Source: CAD feature listing. Evaluate the final solid. Frame: model axes, mm. A direction names the side the tool comes from. Round coordinates to 2 decimals unless told otherwise and drop trailing zeros. Order: outer loops, then holes, each group sorted by start corner. A loop starts at its lowest first (then second) coordinate and runs counter-clockwise, first axis right, second up. Notation, with made-up numbers: (87, 38.5) -> (125, 38.5) arc R19 ccw to (125, 59.5) -> close; hole circle Ø4 at (-3, 65). An arc over 180 degrees is marked (long way). Use a Markdown table: item, result. Add a question column.
```python
from build123d import *

# Parameters (mm, degrees)
CUT_EXTRUDE3_START = 95.1
CUT_EXTRUDE3_DEPTH = 26.1
CIRPATTERN1_COUNT  = 3


with BuildPart() as part:
    # Sketch2 → Revolve1 (revolve)
    with BuildSketch(Plane(origin=(0, 0, 0), x_dir=(0, 0, -1), z_dir=(1, 0, 0)), mode=Mode.PRIVATE) as revolve1_sk:
        Polygon((-172, 135), (172, 135), (172, 120), (426, 120), (426, 0), (0, 0), (-426, 0), (-426, 120), (-172, 120), align=None)
    revolve(revolve1_sk.sketch.rotate(Axis((0, 0, 564.378028921), (0, 0, -1)), 180), axis=Axis((0, 0, 564.378028921), (0, 0, -1)))

    # Sketch3 → Revolve2 (revolve)
    with BuildSketch(Plane(origin=(0, 0, 0), x_dir=(0, 0, -1), z_dir=(1, 0, 0)), mode=Mode.PRIVATE) as revolve2_sk:
        Polygon((426, -119), (426, -15), (923, -15), (923, -95), (678, -95), (678, -110), (614, -110), (614, -107), (602, -107), (602, -112.85), (454, -119), align=None)
    revolve2 = revolve(revolve2_sk.sketch.rotate(Axis((0, -15, 0), (0, 0, -1)), 270), axis=Axis((0, -15, 0), (0, 0, -1)))

    # Mirror1: Revolve2 across plane
    add(revolve2.mirror(Plane.XY))

    # Sketch5 → Cut-Extrude3 (cut)
    with BuildSketch(Plane(origin=(0, 0, 0), x_dir=(1, 0, 0), z_dir=(0, 1, 0)).offset(CUT_EXTRUDE3_START)):
        with BuildLine():
            Line((9, 742), (9, 614))
            ThreePointArc((9, 614), (0, 605), (-9, 614))
            Line((-9, 614), (-9, 742))
            ThreePointArc((-9, 742), (0, 751), (9, 742))
        make_face()
    cut_extrude3 = extrude(amount=-CUT_EXTRUDE3_DEPTH, mode=Mode.SUBTRACT)

    # Mirror2: Cut-Extrude3 across plane
    add(cut_extrude3.mirror(Plane.XY), mode=Mode.SUBTRACT)

    # Sketch7 → M16 Tapped Hole1 (revolve, cut)
    with BuildSketch(Plane(origin=(-51.961524227, 15, -923), x_dir=(0, 1, 0), z_dir=(1, 0, 0))):
        Polygon((0, 0), (0, 42.206024333), (7, 38), (7, 0), align=None)
    m16_tapped_hole1 = revolve(axis=Axis((-51.961524227, 15, -929.35), (0, 0, 1)), mode=Mode.SUBTRACT)

    # CirPattern1: M16 Tapped Hole1 ×3 about axis
    cirpattern1_axis = Axis((0, -15, 0), (0, 0, 1))
    for i in range(1, CIRPATTERN1_COUNT):
        add(m16_tapped_hole1.rotate(cirpattern1_axis, i * 360 / CIRPATTERN1_COUNT), mode=Mode.SUBTRACT)

    # Mirror3: M16 Tapped Hole1 across plane
    add(m16_tapped_hole1.mirror(Plane.XY), mode=Mode.SUBTRACT)

    # Mirror3 copy 1 sketch → Mirror3 copy 1 (revolve, cut)
    with BuildSketch(Plane(origin=(0, -75, 923), x_dir=(-0.8660254037844387, -0.4999999999999998, 0), z_dir=(-0.4999999999999998, 0.8660254037844387, 0))):
        Polygon((0, 0), (0, -42.206024333), (7, -38), (7, 0), align=None)
    revolve(axis=Axis((0, -75, 929.35), (0, 0, 1)), mode=Mode.SUBTRACT)

    # Mirror3 copy 2 sketch → Mirror3 copy 2 (revolve, cut)
    with BuildSketch(Plane(origin=(51.961524227, 15, 923), x_dir=(0.8660254037844384, -0.5000000000000004, 0), z_dir=(-0.5000000000000004, -0.8660254037844384, 0))):
        Polygon((0, 0), (0, -42.206024333), (7, -38), (7, 0), align=None)
    revolve(axis=Axis((51.961524227, 15, 929.35), (0, 0, 1)), mode=Mode.SUBTRACT)


solid = part.part
```
1) Reachability of faces 1 (the cylindrical face through (43.008, -82.456, 798.785)), 2 (the flat face through (-72, 43, -602)), 3 (the flat face through (1, -16, -923)), 4 (the cylindrical face through (-101.184, -64.511, -300.778)) from +Z, -Z, +X, -X, +Y, -Y: full face, straight path, thin tool, end or side. Return the list, or none.
2) Line query: probe 1 along X at (y, z) = (15, -901); probe 2 along Y at (x, z) = (0, -898.5); probe 3 along Y at (x, z) = (7, -52). Output: solid intervals per line, ascending. Write a range as from..to.
3) Section A-A on z = -732.5. Output: boundary loops of the cut face in (x, y), then the cut area to 3 significant figures.
4) Draft query along Z for faces 5 (the flat face through (-0.6, 89.4, -426)), 6 (the cylindrical face through (-82.531, 48.282, 439.804)), 7 (the flat face through (-36, -100, -614)). Return one class per face: pulls with the +Z half, pulls with the -Z half, needs draft (parallel to the pull), parting line crosses it, or undercut.
5) First-contact query: pin 1 Ø14.5 at (x, z) = (0.5, -637) entering from +Y; pin 2 Ø5.5 at (y, z) = (74, 637.5) entering from -X; pin 3 Ø11 at (x, y) = (0, -75) entering from -Z. Flat tips, straight axial feed; report the tip coordinate or a pass-through.
6) Section B-B on z = 383.5. Output: boundary loops of the cut face in (x, y).
Conclusion:
| question | item | result |
|---|---|---|
| 1 | face 1 | +Z |
| 1 | face 2 | none |
| 1 | face 3 | -Z, +X, -X, +Y, -Y |
| 1 | face 4 | -Z |
| 2 | probe 1 | x = -74.16..-58.96, -44.96..44.96, 58.96..74.16 |
| 2 | probe 2 | y = -95..-82, -68..65 |
| 2 | probe 3 | y = -134.82..134.82 |
| 3 | outline | circle Ø160 at (0, -15) |
| 3 | area | 20,100 mm^2 |
| 4 | face 5 | pulls with the -Z half |
| 4 | face 6 | needs draft |
| 4 | face 7 | undercut |
| 5 | pin 1 | stops at y = 69 |
| 5 | pin 2 | stops at x = -39.82 |
| 5 | pin 3 | stops at z = -884.1 |
| 6 | outline | circle Ø240 at (0, 0) |
